```python
from build123d import *

# Parameters (mm, degrees)
SKETCH1_W           = 8
SKETCH1_H           = 6
BOSS_EXTRUDE1_DEPTH = 1
SKETCH2_R           = 0.15
SKETCH2_R_2         = 0.25
SKETCH2_R_3         = 0.35
CUT_EXTRUDE1_DEPTH  = 2
SKETCH3_W           = 8
SKETCH3_H           = 0.5
CUT_EXTRUDE2_DEPTH  = 7


with BuildPart() as part:
    # Sketch1 → Boss-Extrude1 (new body)
    with BuildSketch(Plane.XY):
        with Locations((4, -3)):
            Rectangle(SKETCH1_W, SKETCH1_H)
    extrude(amount=BOSS_EXTRUDE1_DEPTH)

    # Sketch2 → Cut-Extrude1 (cut)
    with BuildSketch(Plane.XY.offset(1)):
        with Locations((1, -1.5)):
            Circle(SKETCH2_R)
        with Locations((1, -3)):
            Circle(SKETCH2_R_2)
        with Locations((1, -4.5)):
            Circle(SKETCH2_R_3)
    extrude(amount=-CUT_EXTRUDE1_DEPTH, mode=Mode.SUBTRACT)

    # Sketch3 → Cut-Extrude2 (cut)
    with BuildSketch(Plane.XY.offset(1)):
        with Locations((4, -0.25)):
            Rectangle(SKETCH3_W, SKETCH3_H)
        with Locations((4, -5.75)):
            Rectangle(SKETCH3_W, SKETCH3_H)
    extrude(amount=-CUT_EXTRUDE2_DEPTH, mode=Mode.SUBTRACT)


solid = part.part
```
Input: part model. Units: mm. Frame: model coordinates. Give positions to 0.01 mm unless a question says otherwise; leave off trailing zeros. Order: outer loops, then holes, each group sorted by start corner. A loop starts at its lowest first (then second) coordinate and runs counter-clockwise, first axis right, second up.
1. Cut plane A-A (y = -1.5). Return loops of the section in (x, z), and give its area (3 significant figures).
Computed:
outline: (0, 0) - (0.85, 0) - (0.85, 1) - (0, 1) - close; (1.15, 0) - (8, 0) - (8, 1) - (1.15, 1) - close
area: 7.70 mm2
2. Line query: probe 1 along Y at (x, z) = (1, 0.4); probe 2 along X at (y, z) = (-4.75, 0.2). Output: solid intervals per line, ascending.
Computed:
probe 1: y = -5.5 to -4.85, -4.15 to -3.25, -2.75 to -1.65, -1.35 to -0.5
probe 2: x = 0 to 0.76, 1.24 to 8
3. Cut plane B-B (z = 0.25). Return loops of the section in (x, y).
Computed:
outline: (0, -5.5) - (8, -5.5) - (8, -0.5) - (0, -0.5) - close; hole circle Ø0.7 at (1, -4.5); hole circle Ø0.5 at (1, -3); hole circle Ø0.3 at (1, -1.5)
4. Cut plane D-D (y = -3). Return loops of the section in (x, z).
Computed:
outline: (0, 0) - (0.75, 0) - (0.75, 1) - (0, 1) - close; (1.25, 0) - (8, 0) - (8, 1) - (1.25, 1) - close
5. Cut plane C-C (x = 1). Return loops of the section in (y, z).
Computed:
outline: (-5.5, 0) - (-4.85, 0) - (-4.85, 1) - (-5.5, 1) - close; (-4.15, 0) - (-3.25, 0) - (-3.25, 1) - (-4.15, 1) - close; (-2.75, 0) - (-1.65, 0) - (-1.65, 1) - (-2.75, 1) - close; (-1.35, 0) - (-0.5, 0) - (-0.5, 1) - (-1.35, 1) - close
